Could you check a few things on this model? Use its own coordinates, in mm. A direction names the side the tool comes from. Coordinates: 2 decimals unless noted, no trailing zeros. Write each loop counter-clockwise with the first axis right and the second up, starting at its lowest first coordinate (ties: lowest second). Pieces come first, ordered by that corner, then holes.
```python
from build123d import *

# Parameters (mm, degrees)
CHAMFER1_SIZE = 1
CHAMFER2_SIZE = 3


with BuildPart() as part:
    # Sketch2 → Revolve1 (revolve)
    with BuildSketch(Plane.XY, mode=Mode.PRIVATE) as revolve1_sk:
        Polygon((0, 10), (0, 16), (-30, 16), (-30, 22.5), (-40, 22.5), (-40, 16), (-45, 16), (-45, 10), align=None)
    revolve(revolve1_sk.sketch.rotate(Axis((0, 0, 0), (-1, 0, 0)), 90), axis=Axis((0, 0, 0), (-1, 0, 0)))

    # Chamfer1
    chamfer1_edges = [part.edges().sort_by_distance(p)[0] for p in [
        (0, 0, 16),
        (-30, 0, 22.5),
        (-40, 0, 22.5),
        (-45, 0, 10),
        (0, 0, 10),
    ]]
    chamfer(chamfer1_edges, length=CHAMFER1_SIZE)

    # Chamfer2
    chamfer2_edges = [part.edges().sort_by_distance(p)[0] for p in [
        (-45, 0, 16),
    ]]
    chamfer(chamfer2_edges, length=CHAMFER2_SIZE)


solid = part.part
```
1. Please list where these lines run through material, in increasing order: line 1 along Y through (x, z) = (-18, 0); line 2 along X through (y, z) = (-5, 15.5); line 3 along Y through (x, z) = (-33, 4.5).
Verdict:
line 1: y = -16 to -10, 10 to 16
line 2: x = -40 to -30
line 3: y = -22.05 to -8.93, 8.93 to 22.05
2. If we mould it in two halves opening along Y, with no side actions, what happens to faces 1 (the face through (-22, 0, 10)), 2 (the face through (-30, -16, -3)), 3 (the face through (-15.7, 15.62, 3.47))? For each: pulls with the +Y half, pulls with the -Y half, needs draft (parallel to the pull), parting line crosses it, or undercut.
Verdict:
face 1: undercut
face 2: needs draft
face 3: parting line crosses it
3. I want a section at A-A on z = 0. Please give me the cut outline in (x, y).
Verdict:
outline: (-45, -13) - (-42, -16) - (-40, -16) - (-40, -21.5) - (-39, -22.5) - (-31, -22.5) - (-30, -21.5) - (-30, -16) - (-1, -16) - (0, -15) - (0, -11) - (-1, -10) - (-44, -10) - (-45, -11) - close; (-45, 11) - (-44, 10) - (-1, 10) - (0, 11) - (0, 15) - (-1, 16) - (-30, 16) - (-30, 21.5) - (-31, 22.5) - (-39, 22.5) - (-40, 21.5) - (-40, 16) - (-42, 16) - (-45, 13) - close
4. I want a section at C-C on x = -23.5. Please give me the cut outline in (y, z), plus the area to 3 significant figures.
Verdict:
outline: circle Ø32 at (0, 0); hole circle Ø20 at (0, 0)
area: 490 mm2
5. For pin 1 (3 mm diameter, centred on x = -19, y = -12.5, fed in from +Z); pin 2 (1 mm diameter, centred on x = -22.5, y = -15, fed in from -Z); pin 3 (4 mm diameter, centred on x = -36, z = 6.5, fed in from -Y), each with a flat end and sliding along its axis, tell me the tip position at first contact or that it passes through.
Verdict:
pin 1: stops at z = 11.62
pin 2: stops at z = -6.76
pin 3: stops at y = -22.05
6. On a 3-axis mill with a long thin cutter (end or side, diameter ignored), from which of +Z, -Z, +X, -X, +Y, -Y can I reach the whole of each face in a straight line? I mean faces 4 (the face through (-35.056, 19.961, -10.382)), 5 (the face through (-40, -16, 3)). Say none if no direction works.
Verdict:
face 4: +X, -X
face 5: -X
